The model under review builds one solid part; all positions refer to its coordinate system, in mm. Round coordinates to 2 decimals unless told otherwise and drop trailing zeros. Order: outer loops, then holes, each group sorted by start corner. A loop starts at its lowest first (then second) coordinate and runs counter-clockwise, first axis right, second up. Notation, with made-up numbers: (-14.5, 80.5) -> (-5.5, 80.5) arc R35 ccw to (-5.5, 115.5) -> close; hole circle Ø5 at (82, 71.25). An arc over 180 degrees is marked (long way). Put each result on its own line as item: value. Start each with the question number.
from build123d import *

# Parameters (mm, degrees)
SKETCH1_R           = 4
SKETCH1_R_2         = 4.5
BOSS_EXTRUDE1_DEPTH = 19
SKETCH2_R           = 4
SKETCH2_R_2         = 4.5
CUT_EXTRUDE1_DEPTH  = 19


with BuildPart() as part:
    # Sketch1 → Boss-Extrude1 (new body)
    with BuildSketch(Plane.XY):
        Polygon((0, 0), (75, 0), (75, 50), (56, 50), (56, 15), (0, 15), align=None)
        with Locations((65.5, 10)):
            Circle(SKETCH1_R, mode=Mode.SUBTRACT)
        with Locations((65.5, 25)):
            Circle(SKETCH1_R_2, mode=Mode.SUBTRACT)
        with Locations((65.5, 40)):
            Circle(SKETCH1_R, mode=Mode.SUBTRACT)
    extrude(amount=BOSS_EXTRUDE1_DEPTH)

    # Sketch2 → Cut-Extrude1 (cut)
    with BuildSketch(Plane(origin=(0, 15, 0), x_dir=(1, 0, 0), z_dir=(0, 1, 0))):
        with Locations(Location((10, -9.5, 0), (0, 0, 180))):
            Circle(SKETCH2_R)
        with Locations(Location((25, -9.5, 0), (0, 0, 180))):
            Circle(SKETCH2_R_2)
        with Locations(Location((40, -9.5, 0), (0, 0, 180))):
            Circle(SKETCH2_R)
    extrude(amount=-CUT_EXTRUDE1_DEPTH, mode=Mode.SUBTRACT)


solid = part.part
Q1. Take a section at A-A on z = 9.5. Give the boundary of the cut face in (x, y), and give its area (3 significant figures).
Q2. Take a section at D-D on x = 65.5. Give the boundary of the cut face in (y, z).
Q3. Draft analysis for pull direction X (two halves, no side actions). For faces 1 (the face through (56, 33, 9)), 2 (the face through (43.2, 7.6, 7.1)), 3 (the face through (28, 15, 14)), state which applies: +X half, -X half, draft (parallel to the pull), parting line (faces both ways), or undercut.
Q4. Clearance check with a flat-ended pin moving along its axis: pin 1 Ø10.5 at (x, z) = (40, 9.5) entering from +Y. State where the tip first meets the part, or that it passes through.
Q5. Take a section at B-B on x = 40. Give the boundary of the cut face in (y, z), and give its area (3 significant figures).
Q6. Take a section at C-C on y = 5. Give the boundary of the cut face in (x, z), and give its area (3 significant figures).
Q7. Wall thickness on probe 1 along Y at (x, z) = (65.5, 10.75); probe 2 along Z at (x, y) = (25, 3.5); probe 3 along X at (y, z) = (9, 7.25): over which ranges is each line inside the solid? List them lowest first. Write a range as [from, to].
Calculated:
1. outline: (0, 0) -> (6, 0) -> (6, 15) -> (0, 15) -> close; (14, 0) -> (20.5, 0) -> (20.5, 15) -> (14, 15) -> close; (29.5, 0) -> (36, 0) -> (36, 15) -> (29.5, 15) -> close; (44, 0) -> (75, 0) -> (75, 50) -> (56, 50) -> (56, 15) -> (44, 15) -> close; hole circle Ø9 at (65.5, 25); hole circle Ø8 at (65.5, 10); hole circle Ø8 at (65.5, 40)
1. area: 1,250 mm²
2. outline: (0, 0) -> (6, 0) -> (6, 19) -> (0, 19) -> close; (14, 0) -> (20.5, 0) -> (20.5, 19) -> (14, 19) -> close; (29.5, 0) -> (36, 0) -> (36, 19) -> (29.5, 19) -> close; (44, 0) -> (50, 0) -> (50, 19) -> (44, 19) -> close
3. face 1: -X half
3. face 2: undercut
3. face 3: draft
4. pin 1: stops at y = 15
5. outline: (0, 0) -> (15, 0) -> (15, 5.5) -> (0, 5.5) -> close; (0, 13.5) -> (15, 13.5) -> (15, 19) -> (0, 19) -> close
5. area: 165 mm²
6. outline: (0, 0) -> (75, 0) -> (75, 19) -> (0, 19) -> close; hole circle Ø8 at (10, 9.5); hole circle Ø9 at (25, 9.5); hole circle Ø8 at (40, 9.5)
6. area: 1,260 mm²
7. probe 1: y = [0, 6], [14, 20.5], [29.5, 36], [44, 50]
7. probe 2: z = [0, 5], [14, 19]
7. probe 3: x = [0, 6.69], [13.31, 21.1], [28.9, 36.69], [43.31, 61.63], [69.37, 75]
